from build123d import *

# Parameters (mm, degrees)
FLANGE_OUTLINE_120_R                 = 60
FLANGE_DISC_DEPTH                    = 10
CENTRE_BORE_PROFILE_20_R             = 10
CENTRE_BORE_20_DEPTH                 = 10
SEED_HOLE_PROFILE_10_R               = 5
SEED_HOLE_10_DEPTH                   = 10
SEED_HOLE_CIRCULAR_PATTERN_6X_COUNT  = 6
RADIAL_HOLE_ROW_3X_COUNT             = 3
RADIAL_HOLE_ROW_3X_PITCH             = 15
RADIAL_HOLE_ROWS_6X_COPY_1_SKETCH_R  = 5
RADIAL_HOLE_ROWS_6X_COPY_1_DEPTH     = 10
RADIAL_HOLE_ROWS_6X_COPY_2_SKETCH_R  = 5
RADIAL_HOLE_ROWS_6X_COPY_2_DEPTH     = 10
RADIAL_HOLE_ROWS_6X_COPY_3_SKETCH_R  = 5
RADIAL_HOLE_ROWS_6X_COPY_3_DEPTH     = 10
RADIAL_HOLE_ROWS_6X_COPY_4_SKETCH_R  = 5
RADIAL_HOLE_ROWS_6X_COPY_4_DEPTH     = 10
RADIAL_HOLE_ROWS_6X_COPY_5_SKETCH_R  = 5
RADIAL_HOLE_ROWS_6X_COPY_5_DEPTH     = 10
RADIAL_HOLE_ROWS_6X_COPY_6_SKETCH_R  = 5
RADIAL_HOLE_ROWS_6X_COPY_6_DEPTH     = 10
RADIAL_HOLE_ROWS_6X_COPY_7_SKETCH_R  = 5
RADIAL_HOLE_ROWS_6X_COPY_7_DEPTH     = 10
RADIAL_HOLE_ROWS_6X_COPY_8_SKETCH_R  = 5
RADIAL_HOLE_ROWS_6X_COPY_8_DEPTH     = 10
RADIAL_HOLE_ROWS_6X_COPY_9_SKETCH_R  = 5
RADIAL_HOLE_ROWS_6X_COPY_9_DEPTH     = 10
RADIAL_HOLE_ROWS_6X_COPY_10_SKETCH_R = 5
RADIAL_HOLE_ROWS_6X_COPY_10_DEPTH    = 10
RADIAL_HOLE_ROWS_6X_COPY_11_SKETCH_R = 5
RADIAL_HOLE_ROWS_6X_COPY_11_DEPTH    = 10
RADIAL_HOLE_ROWS_6X_COPY_12_SKETCH_R = 5
RADIAL_HOLE_ROWS_6X_COPY_12_DEPTH    = 10
RADIAL_HOLE_ROWS_6X_COPY_13_SKETCH_R = 5
RADIAL_HOLE_ROWS_6X_COPY_13_DEPTH    = 10
RADIAL_HOLE_ROWS_6X_COPY_14_SKETCH_R = 5
RADIAL_HOLE_ROWS_6X_COPY_14_DEPTH    = 10
RADIAL_HOLE_ROWS_6X_COPY_15_SKETCH_R = 5
RADIAL_HOLE_ROWS_6X_COPY_15_DEPTH    = 10


with BuildPart() as part:
    # Flange Outline Ø120 → Flange Disc (new body)
    with BuildSketch(Plane.XY):
        Circle(FLANGE_OUTLINE_120_R)
    extrude(amount=FLANGE_DISC_DEPTH)

    # Centre Bore Profile Ø20 → Centre Bore Ø20 (cut)
    with BuildSketch(Plane.XY.offset(10)):
        Circle(CENTRE_BORE_PROFILE_20_R)
    extrude(amount=-CENTRE_BORE_20_DEPTH, mode=Mode.SUBTRACT)

    # Seed Hole Profile Ø10 → Seed Hole Ø10 (cut)
    with BuildSketch(Plane.XY.offset(10)):
        with Locations((20, 0)):
            Circle(SEED_HOLE_PROFILE_10_R)
    seed_hole_10 = extrude(amount=-SEED_HOLE_10_DEPTH, mode=Mode.SUBTRACT)

    # Seed Hole Circular Pattern 6x: Seed Hole Ø10 ×6 about axis
    seed_hole_circular_pattern_6x_axis = Axis((0, 0, 0), (0, 0, 1))
    for i in range(1, SEED_HOLE_CIRCULAR_PATTERN_6X_COUNT):
        add(seed_hole_10.rotate(seed_hole_circular_pattern_6x_axis, i * 360 / SEED_HOLE_CIRCULAR_PATTERN_6X_COUNT), mode=Mode.SUBTRACT)

    # Radial Hole Row 3x: Seed Hole Ø10 ×3
    with Locations(*[(i * RADIAL_HOLE_ROW_3X_PITCH, 0, 0) for i in range(1, RADIAL_HOLE_ROW_3X_COUNT)]):
        add(seed_hole_10, mode=Mode.SUBTRACT)

    # Radial Hole Rows 6x copy 1 sketch → Radial Hole Rows 6x copy 1 (cut)
    with BuildSketch(Plane(origin=(7.5, 12.990381057, 10), x_dir=(0.5000000000000001, 0.8660254037844386, 0), z_dir=(0, 0, 1))):
        with Locations((20, 0)):
            Circle(RADIAL_HOLE_ROWS_6X_COPY_1_SKETCH_R)
    extrude(amount=-RADIAL_HOLE_ROWS_6X_COPY_1_DEPTH, mode=Mode.SUBTRACT)

    # Radial Hole Rows 6x copy 2 sketch → Radial Hole Rows 6x copy 2 (cut)
    with BuildSketch(Plane(origin=(-7.5, 12.990381057, 10), x_dir=(-0.4999999999999998, 0.8660254037844387, 0), z_dir=(0, 0, 1))):
        with Locations((20, 0)):
            Circle(RADIAL_HOLE_ROWS_6X_COPY_2_SKETCH_R)
    extrude(amount=-RADIAL_HOLE_ROWS_6X_COPY_2_DEPTH, mode=Mode.SUBTRACT)

    # Radial Hole Rows 6x copy 3 sketch → Radial Hole Rows 6x copy 3 (cut)
    with BuildSketch(Plane(origin=(-15, 0, 10), x_dir=(-1, 0, 0), z_dir=(0, 0, 1))):
        with Locations((20, 0)):
            Circle(RADIAL_HOLE_ROWS_6X_COPY_3_SKETCH_R)
    extrude(amount=-RADIAL_HOLE_ROWS_6X_COPY_3_DEPTH, mode=Mode.SUBTRACT)

    # Radial Hole Rows 6x copy 4 sketch → Radial Hole Rows 6x copy 4 (cut)
    with BuildSketch(Plane(origin=(-7.5, -12.990381057, 10), x_dir=(-0.5000000000000004, -0.8660254037844384, 0), z_dir=(0, 0, 1))):
        with Locations((20, 0)):
            Circle(RADIAL_HOLE_ROWS_6X_COPY_4_SKETCH_R)
    extrude(amount=-RADIAL_HOLE_ROWS_6X_COPY_4_DEPTH, mode=Mode.SUBTRACT)

    # Radial Hole Rows 6x copy 5 sketch → Radial Hole Rows 6x copy 5 (cut)
    with BuildSketch(Plane(origin=(7.5, -12.990381057, 10), x_dir=(0.5000000000000001, -0.8660254037844386, 0), z_dir=(0, 0, 1))):
        with Locations((20, 0)):
            Circle(RADIAL_HOLE_ROWS_6X_COPY_5_SKETCH_R)
    extrude(amount=-RADIAL_HOLE_ROWS_6X_COPY_5_DEPTH, mode=Mode.SUBTRACT)

    # Radial Hole Rows 6x copy 6 sketch → Radial Hole Rows 6x copy 6 (cut)
    with BuildSketch(Plane(origin=(15, 25.980762114, 10), x_dir=(0.5000000000000001, 0.8660254037844386, 0), z_dir=(0, 0, 1))):
        with Locations((20, 0)):
            Circle(RADIAL_HOLE_ROWS_6X_COPY_6_SKETCH_R)
    extrude(amount=-RADIAL_HOLE_ROWS_6X_COPY_6_DEPTH, mode=Mode.SUBTRACT)

    # Radial Hole Rows 6x copy 7 sketch → Radial Hole Rows 6x copy 7 (cut)
    with BuildSketch(Plane(origin=(-15, 25.980762114, 10), x_dir=(-0.4999999999999998, 0.8660254037844387, 0), z_dir=(0, 0, 1))):
        with Locations((20, 0)):
            Circle(RADIAL_HOLE_ROWS_6X_COPY_7_SKETCH_R)
    extrude(amount=-RADIAL_HOLE_ROWS_6X_COPY_7_DEPTH, mode=Mode.SUBTRACT)

    # Radial Hole Rows 6x copy 8 sketch → Radial Hole Rows 6x copy 8 (cut)
    with BuildSketch(Plane(origin=(-30, 0, 10), x_dir=(-1, 0, 0), z_dir=(0, 0, 1))):
        with Locations((20, 0)):
            Circle(RADIAL_HOLE_ROWS_6X_COPY_8_SKETCH_R)
    extrude(amount=-RADIAL_HOLE_ROWS_6X_COPY_8_DEPTH, mode=Mode.SUBTRACT)

    # Radial Hole Rows 6x copy 9 sketch → Radial Hole Rows 6x copy 9 (cut)
    with BuildSketch(Plane(origin=(-15, -25.980762114, 10), x_dir=(-0.5000000000000004, -0.8660254037844384, 0), z_dir=(0, 0, 1))):
        with Locations((20, 0)):
            Circle(RADIAL_HOLE_ROWS_6X_COPY_9_SKETCH_R)
    extrude(amount=-RADIAL_HOLE_ROWS_6X_COPY_9_DEPTH, mode=Mode.SUBTRACT)

    # Radial Hole Rows 6x copy 10 sketch → Radial Hole Rows 6x copy 10 (cut)
    with BuildSketch(Plane(origin=(15, -25.980762114, 10), x_dir=(0.5000000000000001, -0.8660254037844386, 0), z_dir=(0, 0, 1))):
        with Locations((20, 0)):
            Circle(RADIAL_HOLE_ROWS_6X_COPY_10_SKETCH_R)
    extrude(amount=-RADIAL_HOLE_ROWS_6X_COPY_10_DEPTH, mode=Mode.SUBTRACT)

    # Radial Hole Rows 6x copy 11 sketch → Radial Hole Rows 6x copy 11 (cut)
    with BuildSketch(Plane(origin=(0, 0, 10), x_dir=(0.5000000000000001, 0.8660254037844386, 0), z_dir=(0, 0, 1))):
        with Locations((20, 0)):
            Circle(RADIAL_HOLE_ROWS_6X_COPY_11_SKETCH_R)
    extrude(amount=-RADIAL_HOLE_ROWS_6X_COPY_11_DEPTH, mode=Mode.SUBTRACT)

    # Radial Hole Rows 6x copy 12 sketch → Radial Hole Rows 6x copy 12 (cut)
    with BuildSketch(Plane(origin=(0, 0, 10), x_dir=(-0.4999999999999998, 0.8660254037844387, 0), z_dir=(0, 0, 1))):
        with Locations((20, 0)):
            Circle(RADIAL_HOLE_ROWS_6X_COPY_12_SKETCH_R)
    extrude(amount=-RADIAL_HOLE_ROWS_6X_COPY_12_DEPTH, mode=Mode.SUBTRACT)

    # Radial Hole Rows 6x copy 13 sketch → Radial Hole Rows 6x copy 13 (cut)
    with BuildSketch(Plane(origin=(0, 0, 10), x_dir=(-1, 0, 0), z_dir=(0, 0, 1))):
        with Locations((20, 0)):
            Circle(RADIAL_HOLE_ROWS_6X_COPY_13_SKETCH_R)
    extrude(amount=-RADIAL_HOLE_ROWS_6X_COPY_13_DEPTH, mode=Mode.SUBTRACT)

    # Radial Hole Rows 6x copy 14 sketch → Radial Hole Rows 6x copy 14 (cut)
    with BuildSketch(Plane(origin=(0, 0, 10), x_dir=(-0.5000000000000004, -0.8660254037844384, 0), z_dir=(0, 0, 1))):
        with Locations((20, 0)):
            Circle(RADIAL_HOLE_ROWS_6X_COPY_14_SKETCH_R)
    extrude(amount=-RADIAL_HOLE_ROWS_6X_COPY_14_DEPTH, mode=Mode.SUBTRACT)

    # Radial Hole Rows 6x copy 15 sketch → Radial Hole Rows 6x copy 15 (cut)
    with BuildSketch(Plane(origin=(0, 0, 10), x_dir=(0.5000000000000001, -0.8660254037844386, 0), z_dir=(0, 0, 1))):
        with Locations((20, 0)):
            Circle(RADIAL_HOLE_ROWS_6X_COPY_15_SKETCH_R)
    extrude(amount=-RADIAL_HOLE_ROWS_6X_COPY_15_DEPTH, mode=Mode.SUBTRACT)


solid = part.part
The model under review builds one solid part; all positions refer to its coordinate system, in mm. Give positions to 0.01 mm unless a question says otherwise; leave off trailing zeros. Order: outer loops, then holes, each group sorted by start corner. A loop starts at its lowest first (then second) coordinate and runs counter-clockwise, first axis right, second up. Notation, with made-up numbers: M 41.5,-5 L 55.5,-5 A33 ccw 55.5,26 Z; hole C -12.5,-19.5 d4. An arc over 180 degrees is marked long. One line per question, with ' | ' between items. Start each with the question number.
1) Consider section C-C, the plane y = 28.5. Give the boundary of the cut face in (x, z).
2) Mouldability with a two-part tool opening along X and no side actions: class faces 1 (the face through (30, 0, 5)), 2 (the face through (-1, -12, 10)) as pulls with the +X half, pulls with the -X half, needs draft (parallel to the pull), parting line crosses it, or undercut.
3) Consider section B-B, the plane x = 0. Give the boundary of the cut face in (y, z).
4) Clearance check with flat-ended pins moving along their axes: P1, Ø12, axis at x = 0, y = 0, coming from the +Z side; P2, Ø6, axis at y = -29.5, z = 7, coming from the -X side; P3, Ø4, axis at y = 15, z = 4.5, coming from the -X side; P4, Ø1.5, axis at y = -18.5, z = 4, coming from the -X side. State where each tip first meets the part, or that it passes through.
5) Wall thickness on L1, parallel to X at y = 33.5, z = 4; L2, parallel to X at y = -16, z = 5; L3, parallel to Y at x = 10.5, z = 9.5: over which ranges is each line inside the solid? List them lowest first. Write a range as from..to.
6) Consider section A-A, the plane y = 0. State how many separate pieces and enclosed holes the cut face has, then the cut area to 3 significant figures.
Found:
1) outline: M -52.8,0 L -22.16,0 L -22.16,10 L -52.8,10 Z; M -12.84,0 L 12.84,0 L 12.84,10 L -12.84,10 Z; M 22.16,0 L 52.8,0 L 52.8,10 L 22.16,10 Z
2) face 1: undercut | face 2: needs draft
3) outline: M -60,0 L -10,0 L -10,10 L -60,10 Z; M 10,0 L 60,0 L 60,10 L 10,10 Z
4) P1: passes through | P2: stops at x = -53.83 | P3: stops at x = -58.57 | P4: stops at x = -57.31
5) L1: x = -49.78..-21.35, -13.65..13.65, 21.35..49.78 | L2: x = -57.83..-14.82, -5.18..5.18, 14.82..57.83 | L3: y = -59.07..-22.3, -12.35..12.35, 22.3..59.07
6) separate pieces: 8 | enclosed holes: 0 | area: 400 mm²
